Model file for the job. Use its own axes, mm. Give positions to 0.01 mm unless a question says otherwise; leave off trailing zeros. Loops run counter-clockwise (first coordinate to the right, second up) from the corner with the lowest first, then second, coordinate; pieces in that order, holes last. Notation, with made-up numbers: M -17.75,-14 L 0.25,-14 A17 cw 0.25,3 Z; hole C 35,26 d7. An arc over 180 degrees is marked long. Answer in a Markdown table with one row per item.
```python
from build123d import *

# Parameters (mm, degrees)
SKETCH1_R                      = 111.125
SKETCH1_R_2                    = 84.2
BOSS_EXTRUDE1_DEPTH            = 0.79375
F_9_16_0_5625_DIAMETER_HOLE1_D = 14.2875
F_9_16_0_5625_DIAMETER_HOLE2_D = 14.2875


with BuildPart() as part:
    # Sketch1 → Boss-Extrude1 (new body)
    with BuildSketch(Plane(origin=(0, 0, 0), x_dir=(1, 0, 0), z_dir=(0, 1, 0))):
        with Locations(Location((0, 0, 0), (0, 0, 270))):
            Circle(SKETCH1_R)
        with Locations(Location((0, 0, 0), (0, 0, 270))):
            Circle(SKETCH1_R_2, mode=Mode.SUBTRACT)
    extrude(amount=BOSS_EXTRUDE1_DEPTH)

    # 9/16 (0.5625) Diameter Hole1 (through all)
    with Locations(Plane(origin=(61.2154, 0.79375, -72.9742), x_dir=(0, 0, 1), z_dir=(0, 1, 0))):
        with Locations((0, 0)):
            f_9_16_0_5625_diameter_hole1 = Hole(F_9_16_0_5625_DIAMETER_HOLE1_D / 2)

    # 9/16 (0.5625) Diameter Hole2 (through all)
    with Locations(Plane(origin=(0, 0, 0), x_dir=(-1, 0, 0), z_dir=(0, -1, 0))):
        with Locations((82.4992, 47.625)):
            f_9_16_0_5625_diameter_hole2 = Hole(F_9_16_0_5625_DIAMETER_HOLE2_D / 2)

    # Mirror1: 9/16 (0.5625) Diameter Hole1, 9/16 (0.5625) Diameter Hole2 across plane
    add(f_9_16_0_5625_diameter_hole1.mirror(Plane.XY), mode=Mode.SUBTRACT)
    add(f_9_16_0_5625_diameter_hole2.mirror(Plane.XY), mode=Mode.SUBTRACT)


solid = part.part
```
Q1. Saw through at D-D (y = 0.4). Give the number of separate pieces and of enclosed holes in the cut face, and give its area (3 significant figures).
Reported:
| item | result |
|---|---|
| separate pieces | 1 |
| enclosed holes | 5 |
| area | 15,900 mm² |
Q2. Saw through at B-B (z = 0). Give the cut face in (x, y) (3 decimals), and give its area (3 significant figures).
Reported:
| item | result |
|---|---|
| outline | M -111.125,0 L -84.2,0 L -84.2,0.794 L -111.125,0.794 Z; M 84.2,0 L 111.125,0 L 111.125,0.794 L 84.2,0.794 Z |
| area | 42.7 mm² |
Q3. Saw through at C-C (x = 64.5). Give the cut face in (y, z), and give its area (3 significant figures).
Reported:
| item | result |
|---|---|
| outline | M 0,-90.49 L 0.79,-90.49 L 0.79,-79.32 L 0,-79.32 Z; M 0,-66.63 L 0.79,-66.63 L 0.79,-54.12 L 0,-54.12 Z; M 0,54.12 L 0.79,54.12 L 0.79,66.63 L 0,66.63 Z; M 0,79.32 L 0.79,79.32 L 0.79,90.49 L 0,90.49 Z |
| area | 37.6 mm² |
Q4. Drop a flat-ended pin along its axis: pin 1 (23 mm diameter, centred on x = 61.22, z = 72.97, fed in from +Y). Give the stop position or say it passes through.
Reported:
| item | result |
|---|---|
| pin 1 | y = 0.79 |
Q5. Saw through at A-A (x = 0). Give the cut face in (y, z) (3 decimals).
Reported:
| item | result |
|---|---|
| outline | M 0,-111.125 L 0.794,-111.125 L 0.794,-84.2 L 0,-84.2 Z; M 0,84.2 L 0.794,84.2 L 0.794,111.125 L 0,111.125 Z |
Q6. Mould opens along Z. For faces 1 (the face through (110.18, 0.39, -14.47)), 2 (the face through (66.043, 0.391, 67.709)), 3 (the face through (83, 0.794, -17)) say: released by +Z, released by -Z, zero draft, split by the parting line, or undercut.
Reported:
| item | result |
|---|---|
| face 1 | split by the parting line |
| face 2 | undercut |
| face 3 | zero draft |
Q7. Probe probe 1 along X at (y, z) = (0.1, 76); probe 2 along X at (y, z) = (0.45, -76.5); probe 3 along Z at (x, y) = (-76.5, 0.3). List the from-to ranges inside material, lowest first.
Reported:
| item | result |
|---|---|
| probe 1 | -81.07 to -36.24, 36.24 to 54.74, 67.69 to 81.07 |
| probe 2 | -80.6 to -35.18, 35.18 to 55, 67.43 to 80.6 |
| probe 3 | -80.6 to -51.5, -43.75 to -35.18, 35.18 to 43.75, 51.5 to 80.6 |
